Part print with two shaded views. Sizes in mm from the minimum x, y, z corner. A direction names the side the tool comes from. Round coordinates to 2 decimals unless told otherwise and drop trailing zeros. Order: outer loops, then holes, each group sorted by start corner. A loop starts at its lowest first (then second) coordinate and runs counter-clockwise, first axis right, second up. Notation, with made-up numbers: (62.25, 67.25) -> (120.25, 67.25) arc R9 ccw to (120.25, 84.25) -> close; hole circle Ø4 at (39.5, 75). An arc over 180 degrees is marked (long way). Answer as a JSON object with one key per item and string values.
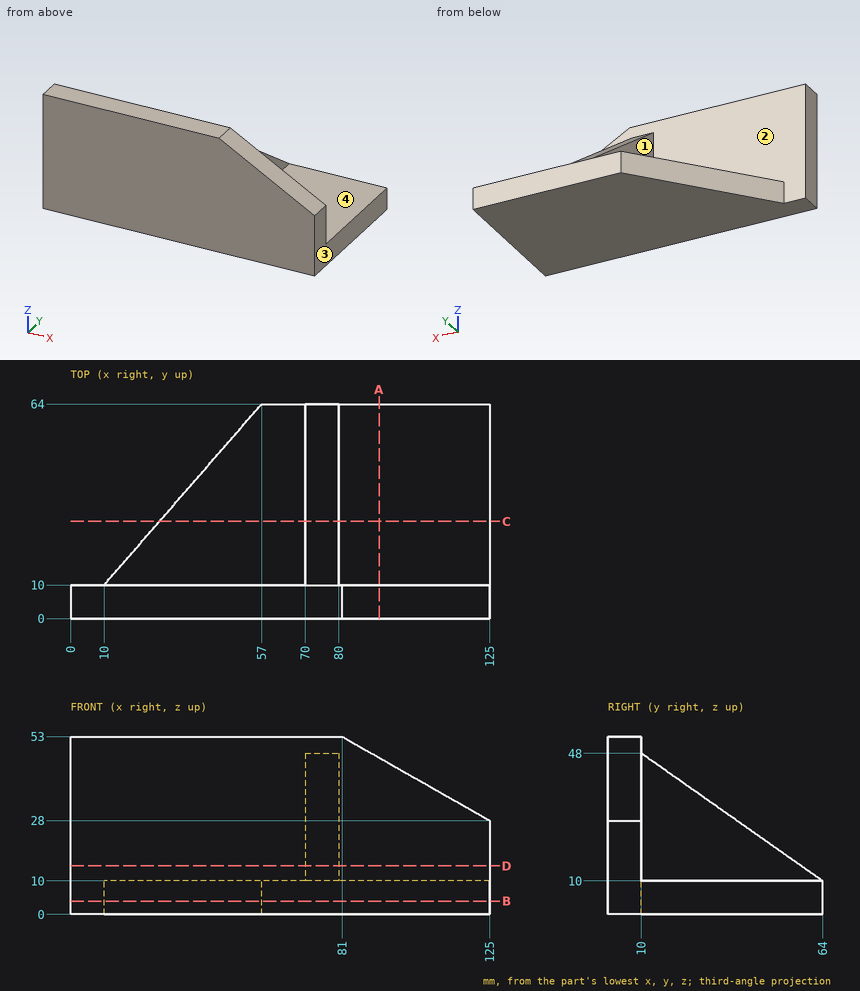
1) Cut at A-A, the plane x = 92. Give the cut face in (y, z), plus the area to 3 significant figures.
Checked values:
{"outline": "(0, 0) -> (64, 0) -> (64, 10) -> (10, 10) -> (10, 46.75) -> (0, 46.75) -> close", "area": "1,010 mm²"}
2) Cut at C-C, the plane y = 29. Give the cut face in (x, z).
Checked values:
{"outline": "(26.54, 0) -> (125, 0) -> (125, 10) -> (80, 10) -> (80, 34.63) -> (70, 34.63) -> (70, 10) -> (26.54, 10) -> close"}
3) Cut at D-D, the plane z = 14.5. Give the cut face in (x, y), plus the area to 3 significant figures.
Checked values:
{"outline": "(0, 0) -> (125, 0) -> (125, 10) -> (80, 10) -> (80, 57.61) -> (70, 57.61) -> (70, 10) -> (0, 10) -> close", "area": "1,730 mm²"}
4) Flat gauge pins, fed straight in: pin 1 Ø2 at (x, z) = (62.5, 44) entering from +Y; pin 2 Ø4 at (y, z) = (17.5, 29.5) entering from -X; pin 3 Ø12 at (y, z) = (18, 19) entering from +X. Where does each tip first touch, or does it go through?
Checked values:
{"pin 1": "stops at y = 10", "pin 2": "stops at x = 70", "pin 3": "stops at x = 80"}
5) Which spindle directions (+Z, -Z, +X, -X, +Y, -Y) get a long thin tool onto all of the face, cutting with end or side? Do the marked faces 1, 2, 3 and 4. Say none if no direction does.
Checked values:
{"face 1": "+Z, -X, +Y", "face 2": "+Z, +Y", "face 3": "+Z, -Z, +X, +Y, -Y", "face 4": "+Z, +X, +Y"}
6) Probe L1, parallel to Y at x = 22.5, z = 40; L2, parallel to X at y = 41, z = 17. List the from-to ranges inside material, lowest first. Write a range as from..to.
Checked values:
{"L1": "y = 0..10", "L2": "x = 70..80"}
7) Cut at B-B, the plane z = 4. Give the cut face in (x, y).
Checked values:
{"outline": "(0, 0) -> (125, 0) -> (125, 64) -> (57, 64) -> (10, 10) -> (0, 10) -> close"}
